Job drawing, mm, ordinate dimensions from the low corner. One solid piece. A direction names the side the tool comes from. Coordinates: 2 decimals unless noted, no trailing zeros. Loops run counter-clockwise (first coordinate to the right, second up) from the corner with the lowest first, then second, coordinate; pieces in that order, holes last. Notation, with made-up numbers: (87.25, 13.5) - (108.25, 13.5) arc R34 ccw to (108.25, 46.5) - close; hole circle Ø8 at (80.5, 16). An arc over 180 degrees is marked (long way). Use a Markdown table: item, result. Add a question column.
1. Band-saw the part on D-D, the plane x = 43. Give the cut face in (y, z).
2. Drop a flat-ended pin along its axis: pin 1 (4.5 mm diameter, centred on x = 20.5, y = 7.5, fed in from -Z). Give the stop position or say it passes through.
3. Wall check: probe 1 along X at (y, z) = (12.75, 5); probe 2 along X at (y, z) = (18.5, 5); probe 3 along Y at (x, z) = (13, 24.75). Give the ranges that are in metal, low to high. Write a range as [from, to].
4. Band-saw the part on C-C, the plane y = 10. Give the cut face in (x, z).
5. Pull direction Z, two halves, no side cores. Call the marked faces 1, 2 and 3: pulls with the +Z half, pulls with the -Z half, needs draft (parallel to the pull), parting line crosses it, or undercut.
6. Band-saw the part on B-B, the plane x = 35. Give the cut face in (y, z).
7. Band-saw the part on A-A, the plane z = 23. Give the cut face in (x, y), plus the area to 3 significant figures.
8. 3-axis set-ups, long thin cutter, end or side, ignore diameter. For the marked faces 4 and 5: which of +Z, -Z, +X, -X, +Y, -Y reach the whole face in a straight line?
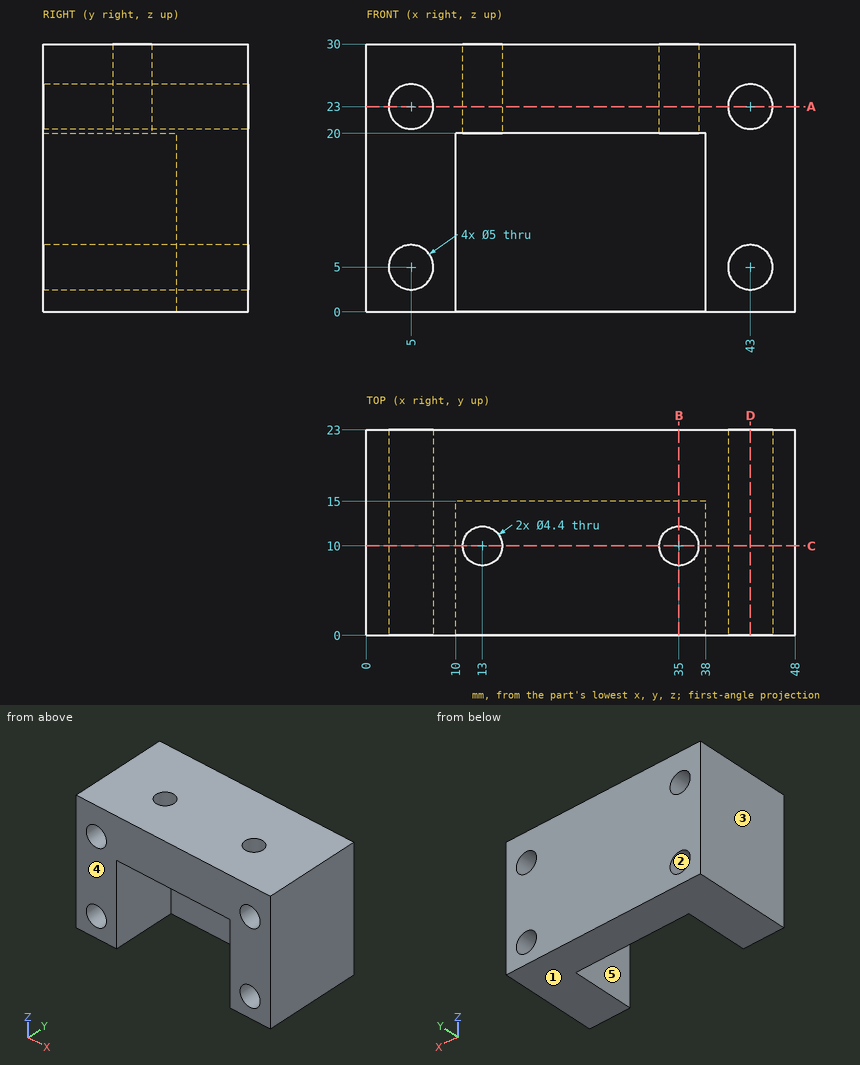
Geometry check:
| question | item | result |
|---|---|---|
| 1 | outline | (0, 0) - (23, 0) - (23, 2.5) - (0, 2.5) - close; (0, 7.5) - (23, 7.5) - (23, 20.5) - (0, 20.5) - close; (0, 25.5) - (23, 25.5) - (23, 30) - (0, 30) - close |
| 2 | pin 1 | stops at z = 20 |
| 3 | probe 1 | x = [0, 2.5], [7.5, 10], [38, 40.5], [45.5, 48] |
| 3 | probe 2 | x = [0, 2.5], [7.5, 40.5], [45.5, 48] |
| 3 | probe 3 | y = [0, 7.8], [12.2, 23] |
| 4 | outline | (0, 0) - (10, 0) - (10, 20) - (10.8, 20) - (10.8, 30) - (0, 30) - close; (15.2, 20) - (32.8, 20) - (32.8, 30) - (15.2, 30) - close; (37.2, 20) - (38, 20) - (38, 0) - (48, 0) - (48, 30) - (37.2, 30) - close; hole circle Ø5 at (5, 5); hole circle Ø5 at (5, 23); hole circle Ø5 at (43, 5); hole circle Ø5 at (43, 23) |
| 5 | face 1 | pulls with the -Z half |
| 5 | face 2 | undercut |
| 5 | face 3 | needs draft |
| 6 | outline | (0, 20) - (7.8, 20) - (7.8, 30) - (0, 30) - close; (12.2, 20) - (15, 20) - (15, 0) - (23, 0) - (23, 30) - (12.2, 30) - close |
| 7 | outline | (0, 0) - (2.5, 0) - (2.5, 23) - (0, 23) - close; (7.5, 0) - (40.5, 0) - (40.5, 23) - (7.5, 23) - close; (45.5, 0) - (48, 0) - (48, 23) - (45.5, 23) - close; hole circle Ø4.4 at (13, 10); hole circle Ø4.4 at (35, 10) |
| 7 | area | 844 mm^2 |
| 8 | face 4 | +Z, -Z, +X, -X, -Y |
| 8 | face 5 | -Z, -Y |
